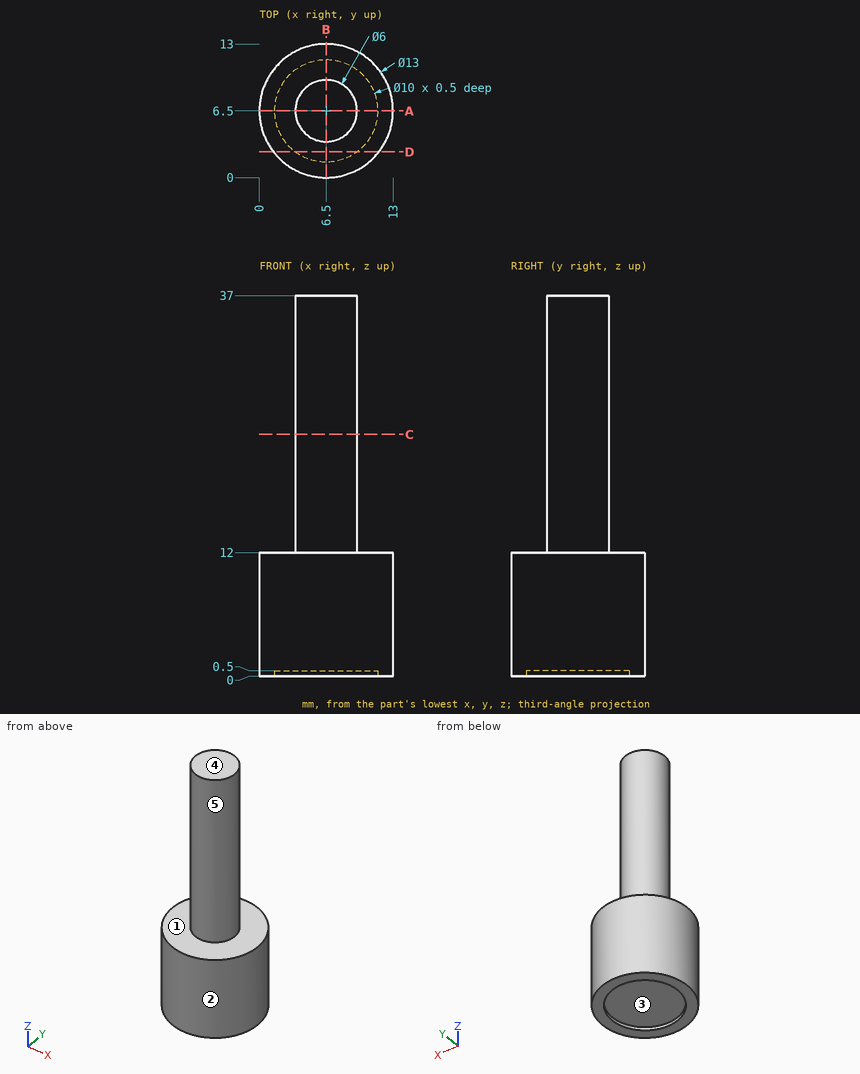
Input: dimensioned drawing with shaded views. Units: mm. Origin: part minimum x, y, z. A direction names the side the tool comes from. Round coordinates to 2 decimals unless told otherwise and drop trailing zeros. Loops run counter-clockwise (first coordinate to the right, second up) from the corner with the lowest first, then second, coordinate; pieces in that order, holes last. Notation, with made-up numbers: M 33,17.25 L 78,17.25 A8 cw 78,23.25 Z; hole C 25.25,44 d1. An arc over 180 degrees is marked long. Return JSON: item names as keys, results as strings. Group by question number.
1. Section query A-A on y = 6.5. Output: boundary loops of the cut face in (x, z).
2. Section query C-C on z = 23.5. Output: boundary loops of the cut face in (x, y), and give its area (3 significant figures).
3. Reachability of the marked faces 1 and 2 from +Z, -Z, +X, -X, +Y, -Y: full face, straight path, thin tool, end or side. Return the list, or none.
4. Material intervals for line 1 along Y through (x, z) = (6.5, 0.25); line 2 along Z through (x, y) = (3.25, 6.25); line 3 along Z through (x, y) = (8.5, 4.5), sorted ascending. Write a range as from..to.
5. Section query D-D on y = 2.5. Output: boundary loops of the cut face in (x, z), and give its area (3 significant figures).
6. Mould query, pull axis Y, two halves, no side actions, for the marked faces 3, 4 and 5. Classes: released by +Y, released by -Y, zero draft, split by the parting line, or undercut.
7. Pin query (flat end, axial travel): pin 1 (1.5 mm diameter, centred on x = 7, z = 28.5, fed in from -Y); pin 2 (6 mm diameter, centred on x = 6.5, y = 6.5, fed in from -Z); pin 3 (1 mm diameter, centred on y = 9.5, z = 11, fed in from +X). Return the tip coordinate at first contact, or that it passes through.
Checks:
{
 "1": {"outline": "M 0,0 L 1.5,0 L 1.5,0.5 L 11.5,0.5 L 11.5,0 L 13,0 L 13,12 L 9.5,12 L 9.5,37 L 3.5,37 L 3.5,12 L 0,12 Z"},
 "2": {"outline": "C 6.5,6.5 d6", "area": "28.3 mm²"},
 "3": {"face 1": "+Z", "face 2": "+Z, -Z"},
 "4": {"line 1": "y = 0..1.5, 11.5..13", "line 2": "z = 0.5..12", "line 3": "z = 0.5..37"},
 "5": {"outline": "M 1.38,0 L 3.5,0 L 3.5,0.5 L 9.5,0.5 L 9.5,0 L 11.62,0 L 11.62,12 L 1.38,12 Z", "area": "120 mm²"},
 "6": {"face 3": "undercut", "face 4": "zero draft", "face 5": "split by the parting line"},
 "7": {"pin 1": "stops at y = 3.5", "pin 2": "stops at z = 0.5", "pin 3": "stops at x = 12.5"}
}
